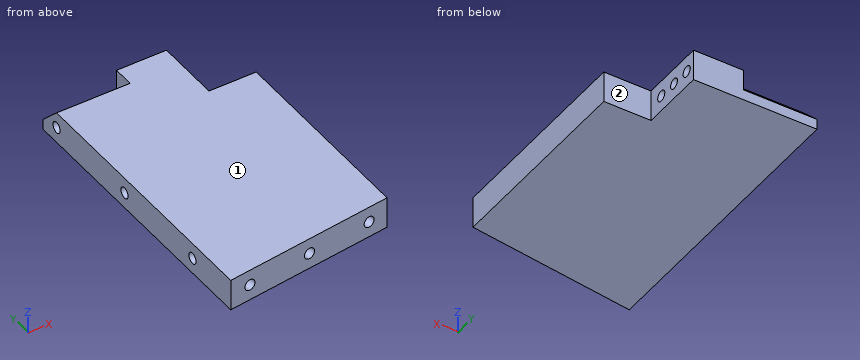
from build123d import *

# Parameters (mm, degrees)
SKETCH1_W                    = 65
SKETCH1_H                    = 12
BOSS_EXTRUDE1_DEPTH          = 51
BOSS_EXTRUDE2_DEPTH          = 12
SKETCH3_W                    = 18
SKETCH3_H                    = 25
CUT_EXTRUDE2_DEPTH           = 69.900909755
M5_TAPPED_HOLE1_D            = 4.2
M5_TAPPED_HOLE1_DEPTH        = 12.4
M5_TAPPED_HOLE1_TIP          = 1.2618073
M5_TAPPED_HOLE2_D            = 4.2
M5_TAPPED_HOLE2_DEPTH        = 12.4
M5_TAPPED_HOLE2_TIP          = 1.2618073
M5_TAPPED_HOLE3_D            = 4.2
M5_TAPPED_HOLE3_DEPTH        = 12.4
M5_TAPPED_HOLE3_TIP          = 1.2618073
CUT_EXTRUDE3_DEPTH           = 28
F_4_0_4_DIAMETER_HOLE1_D     = 4
F_4_0_4_DIAMETER_HOLE1_DEPTH = 8
F_4_0_4_DIAMETER_HOLE1_TIP   = 1.201721238


with BuildPart() as part:
    # Sketch1 → Boss-Extrude1 (new, symmetric)
    with BuildSketch(Plane(origin=(0, 0, 0), x_dir=(1, 0, 0), z_dir=(0, 1, 0))):
        Rectangle(SKETCH1_W, SKETCH1_H)
    extrude(amount=BOSS_EXTRUDE1_DEPTH, both=True)

    # Sketch4 → Boss-Extrude2 (add)
    with BuildSketch(Plane.XY.offset(6)):
        Polygon((-32.5, -51), (32.5, -51), (-32.5, -59.557412343), align=None)
    extrude(amount=-BOSS_EXTRUDE2_DEPTH)

    # Sketch3 → Cut-Extrude2 (cut, through all)
    with BuildSketch(Plane.XY.offset(6)):
        with Locations((23.5, 38.5)):
            Rectangle(SKETCH3_W, SKETCH3_H)
    extrude(amount=-CUT_EXTRUDE2_DEPTH, mode=Mode.SUBTRACT)

    # M5 Tapped Hole1
    with Locations(Plane(origin=(7.153590973, -54.336918053, 0), x_dir=(-0.9914448613738113, -0.13052619222004513, 0), z_dir=(0.13052619222004513, -0.9914448613738113, 0))):
        with Locations((-18.065122191, 0), (6.934877809, 0), (31.934877809, 0)):
            Hole(M5_TAPPED_HOLE1_D / 2, depth=M5_TAPPED_HOLE1_DEPTH)
            with Locations((0, 0, -(M5_TAPPED_HOLE1_DEPTH + M5_TAPPED_HOLE1_TIP / 2))):  # 118° drill point
                Cone(0, M5_TAPPED_HOLE1_D / 2, M5_TAPPED_HOLE1_TIP, mode=Mode.SUBTRACT)

    # M5 Tapped Hole2
    with Locations(Plane.ZY.offset(32.5)):
        with Locations((0, 43), (0, 3), (0, -37)):
            Hole(M5_TAPPED_HOLE2_D / 2, depth=M5_TAPPED_HOLE2_DEPTH)
            with Locations((0, 0, -(M5_TAPPED_HOLE2_DEPTH + M5_TAPPED_HOLE2_TIP / 2))):  # 118° drill point
                Cone(0, M5_TAPPED_HOLE2_D / 2, M5_TAPPED_HOLE2_TIP, mode=Mode.SUBTRACT)

    # M5 Tapped Hole3
    with Locations(Plane(origin=(14.5, 0, 0), x_dir=(0, 0, -1), z_dir=(1, 0, 0))):
        with Locations((0, 47), (0, 32)):
            Hole(M5_TAPPED_HOLE3_D / 2, depth=M5_TAPPED_HOLE3_DEPTH)
            with Locations((0, 0, -(M5_TAPPED_HOLE3_DEPTH + M5_TAPPED_HOLE3_TIP / 2))):  # 118° drill point
                Cone(0, M5_TAPPED_HOLE3_D / 2, M5_TAPPED_HOLE3_TIP, mode=Mode.SUBTRACT)

    # Sketch12 → Cut-Extrude3 (cut)
    with BuildSketch(Plane.ZY.offset(32.5)):
        Polygon((-2, 51), (6, 51), (6, 43), align=None)
    extrude(amount=-CUT_EXTRUDE3_DEPTH, mode=Mode.SUBTRACT)

    # Ø4.0 (4) Diameter Hole1
    with Locations(Plane(origin=(14.5, 0, 0), x_dir=(0, 0, -1), z_dir=(1, 0, 0))):
        with Locations((0, 39.5)):
            Hole(F_4_0_4_DIAMETER_HOLE1_D / 2, depth=F_4_0_4_DIAMETER_HOLE1_DEPTH)
            with Locations((0, 0, -(F_4_0_4_DIAMETER_HOLE1_DEPTH + F_4_0_4_DIAMETER_HOLE1_TIP / 2))):  # 118° drill point
                Cone(0, F_4_0_4_DIAMETER_HOLE1_D / 2, F_4_0_4_DIAMETER_HOLE1_TIP, mode=Mode.SUBTRACT)


solid = part.part
Verification items for the finished model (mm, model axes). Face numbers are marked on the shaded views. A direction names the side the tool comes from. Give positions to 0.01 mm unless a question says otherwise; leave off trailing zeros.
1) Thickness scan on line 1 along Z through (x, y) = (-26.5, 43); line 2 along X through (y, z) = (33.5, 5.5); line 3 along Y through (x, z) = (11, 0). Record the ranges inside material, lowest first.
2) Depth check by flat-ended pin: pin 1 Ø6.5 at (y, z) = (32, 0) entering from +X; pin 2 Ø2.5 at (y, z) = (-37, 0) entering from -X; pin 3 Ø6.5 at (y, z) = (47.5, 3.5) entering from -X; pin 4 Ø1 at (x, z) = (-15.5, 0.5) entering from -Y. Enter the tip coordinate at first touch or a pass-through.
3) Set-up check for the marked faces 1 and 2: record each of +Z, -Z, +X, -X, +Y, -Y from which the full face is reachable in a straight line by a thin tool's end or side.
Answers:
1. line 1: z = -6 to -2.1, 2.1 to 6
1. line 2: x = -32.5 to 14.5
1. line 3: y = -53.83 to 29.9, 34.1 to 37.5, 41.5 to 44.9, 49.1 to 51
2. pin 1: stops at x = 14.5
2. pin 2: stops at x = -19.59
2. pin 3: stops at x = -32.5
2. pin 4: stops at y = -57.39
3. face 1: +Z, +X, -X, +Y, -Y
3. face 2: +Z, -Z, +X, +Y
